from build123d import *

# Parameters (mm, degrees)
EXTRUDE_1_DEPTH              = 17.5
CUT_EXTRUDE_1_REACH          = 59.066
SKETCH_2_R                   = 2
CHAMFER_1_SIZE               = 2
F_6_0MM_1_D                  = 6
F_6_0MM_1_DEPTH              = 15
F_6_0MM_1_TIP                = 1.802581857
HOLE_WIZARD_M6_1_D           = 6.6
HOLE_WIZARD_M6_1_CBORE_D     = 11
HOLE_WIZARD_M6_1_CBORE_DEPTH = 6.8
HOLE_WIZARD_M4_1_D           = 3.3
HOLE_WIZARD_M4_1_DEPTH       = 18.5
HOLE_WIZARD_M4_1_TIP         = 0.991420021


with BuildPart() as part:
    # 草图1 → 凸台-拉伸1 (new, symmetric)
    with BuildSketch(Plane(origin=(0, 0, 0), x_dir=(1, 0, 0), z_dir=(0, 1, 0))):
        Polygon((-35, 0), (35, 0), (35, 28.4), (22.5, 28.4), (22.5, 18.4), (-22.5, 18.4), (-22.5, 28.4), (-35, 28.4), align=None)
    extrude(amount=EXTRUDE_1_DEPTH, both=True)

    # 草图2 → 切除-拉伸1 (cut, up to next)
    with BuildSketch(Plane(origin=(0, 17.5, 0), x_dir=(1, 0, 0), z_dir=(0, 1, 0)), mode=Mode.PRIVATE) as cut_extrude_1_sk1:
        with Locations((20.5, 18.4)):
            Circle(SKETCH_2_R)
    cut_extrude_1_tool1 = extrude(cut_extrude_1_sk1.sketch, amount=-CUT_EXTRUDE_1_REACH, mode=Mode.PRIVATE) & part.part
    # 草图2 → 切除-拉伸1 (cut, up to next)
    with BuildSketch(Plane(origin=(0, 17.5, 0), x_dir=(1, 0, 0), z_dir=(0, 1, 0)), mode=Mode.PRIVATE) as cut_extrude_1_sk2:
        with Locations((-20.5, 18.4)):
            Circle(SKETCH_2_R)
    cut_extrude_1_tool2 = extrude(cut_extrude_1_sk2.sketch, amount=-CUT_EXTRUDE_1_REACH, mode=Mode.PRIVATE) & part.part
    add(cut_extrude_1_tool1.solids().sort_by_distance((20.5, 17.5, -18.4))[0], mode=Mode.SUBTRACT)
    add(cut_extrude_1_tool2.solids().sort_by_distance((-20.5, 17.5, -18.4))[0], mode=Mode.SUBTRACT)

    # 倒角1
    chamfer_1_edges = [part.edges().sort_by_distance(p)[0] for p in [
        (35, -17.5, -14.2),
        (-35, -17.5, -14.2),
        (35, 17.5, -14.2),
        (-35, 17.5, -14.2),
    ]]
    chamfer(chamfer_1_edges, length=CHAMFER_1_SIZE)

    # Ø6.0mm 暗销孔1
    with Locations(Plane.XY):
        with Locations((-15, 0), (15, 0)):
            Hole(F_6_0MM_1_D / 2, depth=F_6_0MM_1_DEPTH)
            with Locations((0, 0, -(F_6_0MM_1_DEPTH + F_6_0MM_1_TIP / 2))):  # 118° drill point
                Cone(0, F_6_0MM_1_D / 2, F_6_0MM_1_TIP, mode=Mode.SUBTRACT)

    # M6 六角圆柱头螺钉的柱形沉头孔1 (through all)
    with Locations(Plane(origin=(0, 0, -28.4), x_dir=(-1, 0, 0), z_dir=(0, 0, -1))):
        with Locations((-29, 0), (29, 0)):
            CounterBoreHole(HOLE_WIZARD_M6_1_D / 2, HOLE_WIZARD_M6_1_CBORE_D / 2, HOLE_WIZARD_M6_1_CBORE_DEPTH)

    # M4 螺纹孔1
    with Locations(Plane(origin=(0, 0, -28.4), x_dir=(-1, 0, 0), z_dir=(0, 0, -1))):
        with Locations((-29, 12.5), (-29, -12.5), (29, 12.5), (29, -12.5)):
            Hole(HOLE_WIZARD_M4_1_D / 2, depth=HOLE_WIZARD_M4_1_DEPTH)
            with Locations((0, 0, -(HOLE_WIZARD_M4_1_DEPTH + HOLE_WIZARD_M4_1_TIP / 2))):  # 118° drill point
                Cone(0, HOLE_WIZARD_M4_1_D / 2, HOLE_WIZARD_M4_1_TIP, mode=Mode.SUBTRACT)


solid = part.part
Check sheet for the modelled part. Datum: model origin and axes. Units: mm. A direction names the side the tool comes from. Round coordinates to 2 decimals unless told otherwise and drop trailing zeros. Loops run counter-clockwise (first coordinate to the right, second up) from the corner with the lowest first, then second, coordinate; pieces in that order, holes last. Notation, with made-up numbers: M 88,35.5 L 96,35.5 A18 ccw 96,55.5 Z; hole C 7.25,5 d4. An arc over 180 degrees is marked long. One line per question, with ' | ' between items. Start each with the question number.
Item 1: Section check B-B (x = 20.5). Record the boundary of the cut face in (y, z), and give its area (3 significant figures).
Item 2: Section check C-C (x = -3.5). Record the boundary of the cut face in (y, z), and give its area (3 significant figures).
Item 3: Release check for a two-part mould opening along Y. For faces 1 (the face through (34, -16.5, -14)), 2 (the face through (29.286, 12.513, -9.081)), 3 (the face through (0, 17.5, -11)) record: released by +Y, released by -Y, zero draft, split by the parting line, or undercut.
Item 4: Section check A-A (y = -4). Record the boundary of the cut face in (x, z).
Item 5: Set-up check for faces 4 (the face through (0, 0, -18.4)), 5 (the face through (-30.31, -13.5, -19.02)), 6 (the face through (18, 0, -8)): record each of +Z, -Z, +X, -X, +Y, -Y from which the full face is reachable in a straight line by a thin tool's end or side.
Item 6: Scan lines: probe 1 along Y at (x, z) = (29, -20.25); probe 2 along X at (y, z) = (12.5, -19.75); probe 3 along X at (y, z) = (10.5, -20.25). Record each from-to range of solid material in increasing order.
Item 7: Gauge pin test, flat ends, axial feed: pin 1 Ø5.5 at (x, y) = (-31, -1.5) entering from -Z; pin 2 Ø5.5 at (x, y) = (-29, 12.5) entering from +Z; pin 3 Ø12 at (x, y) = (-0.5, 7) entering from -Z. Record the tip position at first contact, or that the pin passes through.
Worked out:
1) outline: M -17.5,-16.4 L 17.5,-16.4 L 17.5,0 L -17.5,0 Z | area: 574 mm^2
2) outline: M -17.5,-18.4 L 17.5,-18.4 L 17.5,0 L -17.5,0 Z | area: 644 mm^2
3) face 1: released by -Y | face 2: undercut | face 3: released by +Y
4) outline: M -35,-28.4 L -32.77,-28.4 L -32.77,-21.6 L -25.23,-21.6 L -25.23,-28.4 L -22.5,-28.4 L -22.5,-18.4 A2 cw -18.5,-18.4 L 18.5,-18.4 A2 cw 22.5,-18.4 L 22.5,-28.4 L 25.23,-28.4 L 25.23,-21.6 L 32.77,-21.6 L 32.77,-28.4 L 35,-28.4 L 35,0 L -35,0 Z
5) face 4: -Z, +Y, -Y | face 5: -Z | face 6: +Z
6) probe 1: -17.5 to -14.15, -10.85 to -3.3, 3.3 to 10.85, 14.15 to 17.5 | probe 2: -35 to -30.65, -27.35 to -22.5, 22.5 to 27.35, 30.65 to 35 | probe 3: -35 to -22.5, 22.5 to 35
7) pin 1: z = -21.6 | pin 2: z = 0 | pin 3: z = -18.4
